Here's how the part is built. I have some questions about the finished solid (model axes, mm). A direction names the side the tool comes from. Give positions to 0.01 mm unless a question says otherwise; leave off trailing zeros. Write each loop counter-clockwise with the first axis right and the second up, starting at its lowest first coordinate (ties: lowest second). Pieces come first, ordered by that corner, then holes. Notation, with made-up numbers: (-1.5, 25.25) -> (24.5, 25.25) arc R15 ccw to (24.5, 31.25) -> close; hole circle Ø4 at (-37.5, 51.25). An arc over 180 degrees is marked (long way). Return JSON: item names as keys, results as strings.
from build123d import *

# Parameters (mm, degrees)
BOSS_EXTRUDE3_DEPTH = 5
BOSS_EXTRUDE4_DEPTH = 8.4
SHELL1_T            = -0.4


with BuildPart() as part:
    # Sketch1 → Boss-Extrude3 (new body)
    with BuildSketch(Plane(origin=(0, 0, 0), x_dir=(1, 0, 0), z_dir=(0, 1, 0))):
        with BuildLine():
            ThreePointArc((0, 2.5), (-1.25, 2.165063509), (-2.165063509, 1.25))
            ThreePointArc((-2.165063509, 1.25), (-2.5, 0), (-2.165063509, -1.25))
            ThreePointArc((-2.165063509, -1.25), (-1.25, -2.165063509), (0, -2.5))
            ThreePointArc((0, -2.5), (1.25, -2.165063509), (2.165063509, -1.25))
            ThreePointArc((2.165063509, -1.25), (2.5, 0), (2.165063509, 1.25))
            ThreePointArc((2.165063509, 1.25), (1.25, 2.165063509), (0, 2.5))
        make_face()
    extrude(amount=BOSS_EXTRUDE3_DEPTH)

    # Sketch2 → Boss-Extrude4 (add)
    with BuildSketch(Plane(origin=(0, 13.4, 0), x_dir=(1, 0, 0), z_dir=(0, 1, 0))):
        Polygon((0, 1.962990915), (-1.7, 0.981495458), (-1.7, -0.981495458), (0, -1.962990915), (1.7, -0.981495458), (1.7, 0.981495458), align=None)
    extrude(amount=-BOSS_EXTRUDE4_DEPTH)

    # Shell1
    shell1_openings = [part.faces().sort_by_distance(p)[0] for p in [
        (0, 13.4, 0),
        (0, 0, 0),
    ]]
    offset(amount=SHELL1_T, openings=shell1_openings, kind=Kind.INTERSECTION)


solid = part.part
1. For pin 1 Ø3 at (y, z) = (5.5, -2) entering from +X; pin 2 Ø0.6 at (y, z) = (9, 0) entering from +X; pin 3 Ø2 at (y, z) = (7, -0.5) entering from -X; pin 4 Ø1.5 at (x, z) = (-0.5, 0) entering from +Y, each with a flat end and sliding along its axis, tell me the tip position at first contact or that it passes through.
Taken from the geometry:
{"pin 1": "stops at x = 2.43", "pin 2": "stops at x = 1.7", "pin 3": "stops at x = -1.7", "pin 4": "passes through"}
2. Suppose I cut it at C-C, the plane z = 0.55. List the corners of the cut face in (x, y) for me, and give its area (3 significant figures).
Taken from the geometry:
{"outline": "(-2.44, 0) -> (-2.03, 0) -> (-2.03, 4.6) -> (-1.3, 4.6) -> (-1.3, 13.4) -> (-1.7, 13.4) -> (-1.7, 5) -> (-2.44, 5) -> close; (1.3, 4.6) -> (2.03, 4.6) -> (2.03, 0) -> (2.44, 0) -> (2.44, 5) -> (1.7, 5) -> (1.7, 13.4) -> (1.3, 13.4) -> close", "area": "11.4 mm²"}
3. Suppose I cut it at A-A, the plane x = -1. List the corners of the cut face in (y, z) for me.
Taken from the geometry:
{"outline": "(0, -2.29) -> (5, -2.29) -> (5, -1.39) -> (13.4, -1.39) -> (13.4, -0.92) -> (4.6, -0.92) -> (4.6, -1.85) -> (0, -1.85) -> close; (0, 1.85) -> (4.6, 1.85) -> (4.6, 0.92) -> (13.4, 0.92) -> (13.4, 1.39) -> (5, 1.39) -> (5, 2.29) -> (0, 2.29) -> close"}
4. If we mould it in two halves opening along Z, with no side actions, what happens to faces 1 (the face through (-2, 5, 0)), 2 (the face through (0.8, 9.3, 1.5)), 3 (the face through (1.3, 9, 0))? For each: released by +Z, released by -Z, zero draft, split by the parting line, or undercut.
Taken from the geometry:
{"face 1": "zero draft", "face 2": "released by +Z", "face 3": "undercut"}
5. Suppose I cut it at B-B, the plane y = 11. List the corners of the cut face in (x, z) for me, and give its area (3 significant figures).
Taken from the geometry:
{"outline": "(-1.7, -0.98) -> (0, -1.96) -> (1.7, -0.98) -> (1.7, 0.98) -> (0, 1.96) -> (-1.7, 0.98) -> close; hole (-1.3, -0.75) -> (0, -1.5) -> (1.3, -0.75) -> (1.3, 0.75) -> (0, 1.5) -> (-1.3, 0.75) -> close", "area": "4.16 mm²"}
6. Suppose I cut it at D-D, the plane x = 1.5. List the corners of the cut face in (y, z) for me, and give its area (3 significant figures).
Taken from the geometry:
{"outline": "(0, -2) -> (5, -2) -> (5, -1.1) -> (13.4, -1.1) -> (13.4, 1.1) -> (5, 1.1) -> (5, 2) -> (0, 2) -> (0, 1.47) -> (4.6, 1.47) -> (4.6, -1.47) -> (0, -1.47) -> close", "area": "24.9 mm²"}
7. Which directions (+Z, -Z, +X, -X, +Y, -Y) give clear straight access to the entire face, cutting with the end or side of a thin tool? Please do faces 4 (the face through (-0.8, 9.3, -1.5)), 5 (the face through (-1.3, 9, 0)), 6 (the face through (1.7, 9, 0)), 7 (the face through (0.862, 9.259, -1.465)).
Taken from the geometry:
{"face 4": "-Z, -X, +Y", "face 5": "+Y, -Y", "face 6": "+Z, -Z, +X, +Y", "face 7": "-Z, +X, +Y"}
8. If I drill on line 1 (X direction, y = 12.75, z = 0.45); line 2 (Y direction, x = -1.65, z = 1.65); line 3 (Z direction, x = 1.4, y = 2.75), over which ranges is the centre line in solid material (lowest first)? Write a range as [from, to].
Taken from the geometry:
{"line 1": "x = [-1.7, -1.3], [1.3, 1.7]", "line 2": "y = [0, 5]", "line 3": "z = [-2.07, -1.57], [1.57, 2.07]"}
